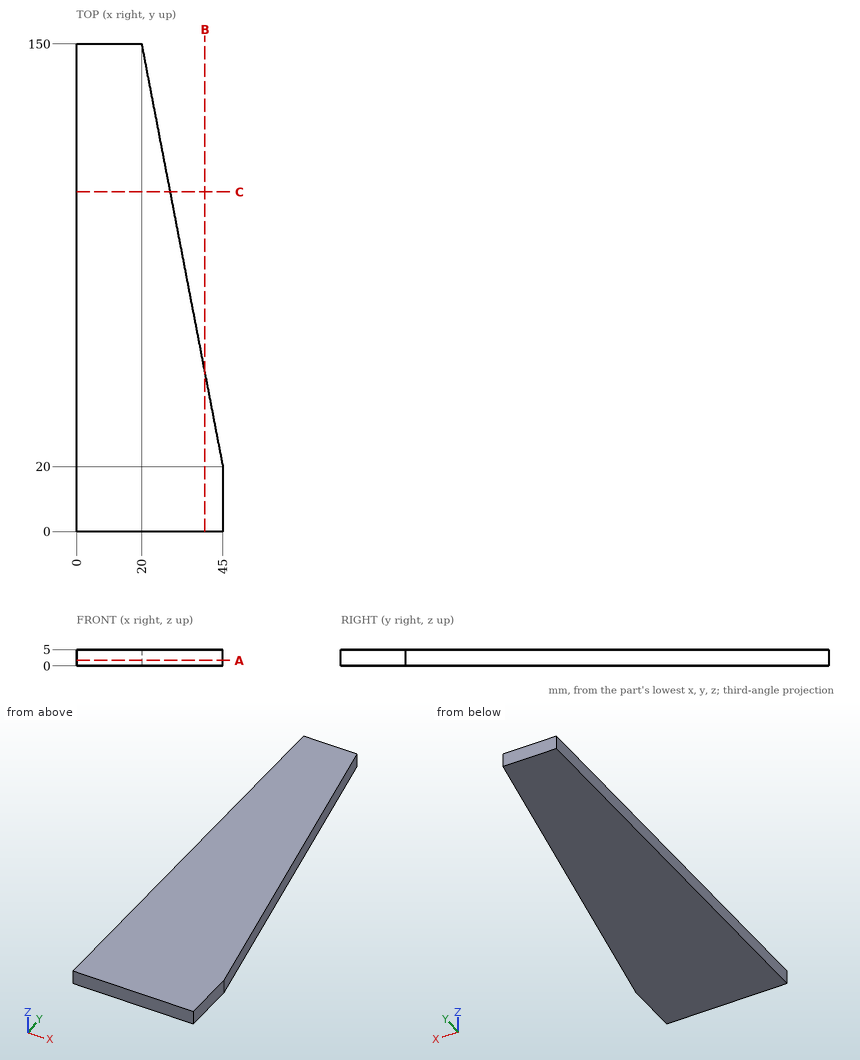
Design review of the part shown in the three views and the two pictorial views. Dimensions are in mm from the part's minimum x, y and z. Give positions to 0.01 mm unless a question says otherwise; leave off trailing zeros. Write each loop counter-clockwise with the first axis right and the second up, starting at its lowest first coordinate (ties: lowest second). Pieces come first, ordered by that corner, then holes. Notation, with made-up numbers: M 24,34 L 34,34 A12 ccw 34,57 Z; hole C 23,72.25 d2. An arc over 180 degrees is marked long. Return JSON: item names as keys, results as strings. Group by question number.
Item 1: Wall thickness on line 1 along X through (y, z) = (74, 3.5); line 2 along X through (y, z) = (65.5, 1): over which ranges is each line inside the solid? List them lowest first.
Item 2: Take a section at B-B (x = 39.5). Give the boundary of the cut face in (y, z).
Item 3: Take a section at A-A (z = 1.75). Give the boundary of the cut face in (x, y), plus the area to 4 significant figures.
Item 4: Clearance check with flat-ended pins moving along their axes: pin 1 Ø1.5 at (y, z) = (83.5, 1.5) entering from +X; pin 2 Ø1.5 at (y, z) = (51.5, 3) entering from +X; pin 3 Ø10 at (x, y) = (35.5, 103) entering from +Z; pin 4 Ø3 at (x, z) = (33, 1.5) entering from -Y. State where each tip first meets the part, or that it passes through.
Item 5: Take a section at C-C (y = 104.5). Give the boundary of the cut face in (x, z), plus the area to 3 significant figures.
Return value:
{
 "1": {"line 1": "x = 0 to 34.62", "line 2": "x = 0 to 36.25"},
 "2": {"outline": "M 0,0 L 48.6,0 L 48.6,5 L 0,5 Z"},
 "3": {"outline": "M 0,0 L 45,0 L 45,20 L 20,150 L 0,150 Z", "area": "5,125 mm2"},
 "4": {"pin 1": "stops at x = 32.93", "pin 2": "stops at x = 39.09", "pin 3": "passes through", "pin 4": "stops at y = 0"},
 "5": {"outline": "M 0,0 L 28.75,0 L 28.75,5 L 0,5 Z", "area": "144 mm2"}
}
